```python
from build123d import *

# Parameters (mm, degrees)
HEX_BODY_25AF_X10_DEPTH = 10
BORE_SKETCH_16_R        = 8
BORE_16_DEPTH           = 10


with BuildPart() as part:
    # Hex Profile Sketch 25AF → Hex Body 25AF x10 (new body)
    with BuildSketch(Plane.XY):
        Polygon((14.43375673, 0), (7.216878365, 12.5), (-7.216878365, 12.5), (-14.43375673, 0), (-7.216878365, -12.5), (7.216878365, -12.5), align=None)
    extrude(amount=HEX_BODY_25AF_X10_DEPTH)

    # Bore Sketch Ø16 → Bore Ø16 (cut)
    with BuildSketch(Plane.XY.offset(10)):
        Circle(BORE_SKETCH_16_R)
    extrude(amount=-BORE_16_DEPTH, mode=Mode.SUBTRACT)


solid = part.part
```
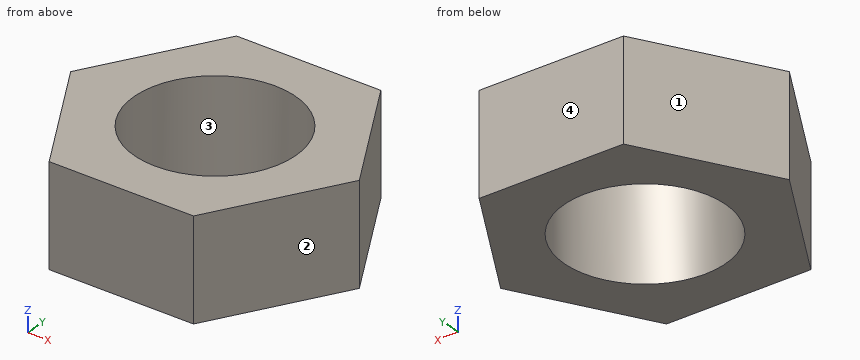
Could you check a few things on this model? Use its own coordinates, in mm. Face numbers are marked on the shaded views. Coordinates: 2 decimals unless noted, no trailing zeros. Order: outer loops, then holes, each group sorted by start corner. A loop starts at its lowest first (then second) coordinate and runs counter-clockwise, first axis right, second up. Notation, with made-up numbers: M 2,66 L 26,66 A18 ccw 26,93 Z; hole C -39.75,-22.75 d3. An arc over 180 degrees is marked long. Use one line per item in the form item = value. Start each with the question number.
1. For pin 1 (3 mm diameter, centred on y = -4.5, z = 7.5, fed in from +X); pin 2 (1.5 mm diameter, centred on x = 3.5, y = -8, fed in from -Z); pin 3 (2 mm diameter, centred on y = -4.5, z = 3, fed in from -X); pin 4 (3 mm diameter, centred on y = 0, z = 4.5, fed in from +X), each with a flat end and sliding along its axis, tell me the tip position at first contact or that it passes through.
2. Please list where these lines run through material, in increasing order: line 1 (Y direction, x = 0, z = 3.25); line 2 (Y direction, x = -4.5, z = 7.5); line 3 (X direction, y = -11.5, z = 8.5).
3. Suppose I cut it at D-D on x = 10.75. Write out the boundary of the cut face in (y, z).
4. We'd pull the mould along X, two halves only. Please class the marked faces 1, 2, 3 and 4: +X half, -X half, draft (parallel to the pull), parting line (faces both ways), or undercut.
5. Suppose I cut it at B-B on y = -7. Write out the boundary of the cut face in (x, z), then the cut area to 3 significant figures.
6. Suppose I cut it at A-A on x = 0. Write out the boundary of the cut face in (y, z), then the cut area to 3 significant figures.
7. Suppose I cut it at C-C on z = 4. Write out the boundary of the cut face in (x, y).
Geometry says:
q1.pin_1 = 12.7
q1.pin_2 = 0
q1.pin_3 = -12.41
q1.pin_4 = 14.43
q2.line_1 = -12.5 to -8, 8 to 12.5
q2.line_2 = -12.5 to -6.61, 6.61 to 12.5
q2.line_3 = -7.79 to 7.79
q3.outline = M -6.38,0 L 6.38,0 L 6.38,10 L -6.38,10 Z
q4.face_1 = -X half
q4.face_2 = +X half
q4.face_3 = undercut
q4.face_4 = draft
q5.outline = M -10.39,0 L -3.87,0 L -3.87,10 L -10.39,10 Z; M 3.87,0 L 10.39,0 L 10.39,10 L 3.87,10 Z
q5.area = 130 mm^2
q6.outline = M -12.5,0 L -8,0 L -8,10 L -12.5,10 Z; M 8,0 L 12.5,0 L 12.5,10 L 8,10 Z
q6.area = 90.0 mm^2
q7.outline = M -14.43,0 L -7.22,-12.5 L 7.22,-12.5 L 14.43,0 L 7.22,12.5 L -7.22,12.5 Z; hole C 0,0 d16
